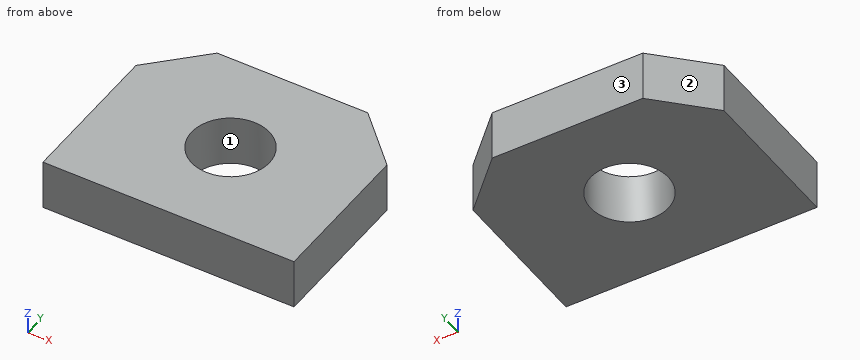
```python
from build123d import *

# Parameters (mm, degrees)
SKETCH1_W              = 50
SKETCH1_H              = 40
BOSS_EXTRUDE1_DEPTH    = 10
CHAMFER1_SIZE          = 10
M18_TAPPED_HOLE1_D     = 15.5
M18_TAPPED_HOLE1_DEPTH = 43.5
M18_TAPPED_HOLE1_TIP   = 4.656669797


with BuildPart() as part:
    # Sketch1 → Boss-Extrude1 (new body)
    with BuildSketch(Plane.XY):
        Rectangle(SKETCH1_W, SKETCH1_H)
    extrude(amount=BOSS_EXTRUDE1_DEPTH)

    # Chamfer1
    chamfer1_edges = [part.edges().sort_by_distance(p)[0] for p in [
        (25, 20, 5),
        (-25, 20, 5),
    ]]
    chamfer(chamfer1_edges, length=CHAMFER1_SIZE)

    # M18 Tapped Hole1
    with Locations(Plane(origin=(0, 0, 0), x_dir=(-1, 0, 0), z_dir=(0, 0, -1))):
        with Locations((0, 0)):
            Hole(M18_TAPPED_HOLE1_D / 2, depth=M18_TAPPED_HOLE1_DEPTH)
            with Locations((0, 0, -(M18_TAPPED_HOLE1_DEPTH + M18_TAPPED_HOLE1_TIP / 2))):  # 118° drill point
                Cone(0, M18_TAPPED_HOLE1_D / 2, M18_TAPPED_HOLE1_TIP, mode=Mode.SUBTRACT)


solid = part.part
```
Verification items for the finished model (mm, model axes). Face numbers are marked on the shaded views. Coordinates: 2 decimals unless noted, no trailing zeros. Order: outer loops, then holes, each group sorted by start corner. A loop starts at its lowest first (then second) coordinate and runs counter-clockwise, first axis right, second up. Notation, with made-up numbers: (63, 17.25) - (115, 17.25) arc R19 ccw to (115, 44.25) - close; hole circle Ø11 at (63.25, 63.5). An arc over 180 degrees is marked (long way). Return JSON: item names as keys, results as strings.
(1) Go/stop test with a flat-tipped pin: pin 1 (1.5 mm diameter, centred on x = -17, z = 3, fed in from +Y). Record where the tip stops, or that it passes through.
Filled sheet:
{"pin 1": "stops at y = 18.75"}
(2) Section check B-B, the plane x = 0. Record the cut outline in (y, z), and give its area (3 significant figures).
Filled sheet:
{"outline": "(-20, 0) - (-7.75, 0) - (-7.75, 10) - (-20, 10) - close; (7.75, 0) - (20, 0) - (20, 10) - (7.75, 10) - close", "area": "245 mm^2"}
(3) Section check C-C, the plane z = 3. Record the cut outline in (x, y).
Filled sheet:
{"outline": "(-25, -20) - (25, -20) - (25, 10) - (15, 20) - (-15, 20) - (-25, 10) - close; hole circle Ø15.5 at (0, 0)"}
(4) Section check A-A, the plane y = 0. Record the cut outline in (x, z), and give its area (3 significant figures).
Filled sheet:
{"outline": "(-25, 0) - (-7.75, 0) - (-7.75, 10) - (-25, 10) - close; (7.75, 0) - (25, 0) - (25, 10) - (7.75, 10) - close", "area": "345 mm^2"}
(5) Section check D-D, the plane x = 18. Record the cut outline in (y, z).
Filled sheet:
{"outline": "(-20, 0) - (17, 0) - (17, 10) - (-20, 10) - close"}
(6) Mould release check, pull along X, two halves, no side actions. Record for the marked faces 1, 2 and 3: pulls with the +X half, pulls with the -X half, needs draft (parallel to the pull), parting line crosses it, or undercut.
Filled sheet:
{"face 1": "undercut", "face 2": "pulls with the -X half", "face 3": "needs draft"}
(7) Thickness scan on line 1 along Y through (x, z) = (0, 5); line 2 along Y through (x, z) = (3, 6.5); line 3 along Y through (x, z) = (-19, 0.75). Record the ranges inside material, lowest first.
Filled sheet:
{"line 1": "y = -20 to -7.75, 7.75 to 20", "line 2": "y = -20 to -7.15, 7.15 to 20", "line 3": "y = -20 to 16"}
